from build123d import *

# Parameters (mm, degrees)
SKETCH1_W           = 140
SKETCH1_H           = 140
BOSS_EXTRUDE1_DEPTH = 34
SKETCH3_R           = 8
CUT_EXTRUDE3_DEPTH  = 105.670912865
CHAMFER1_SIZE       = 5
CHAMFER2_SIZE       = 15
CHAMFER3_SIZE       = 40


with BuildPart() as part:
    # Sketch1 → Boss-Extrude1 (new body)
    with BuildSketch(Plane.XY):
        Rectangle(SKETCH1_W, SKETCH1_H)
    extrude(amount=BOSS_EXTRUDE1_DEPTH)

    # Sketch3 → Cut-Extrude3 (cut, through all)
    with BuildSketch(Plane.XY.offset(34)):
        with Locations((0, -50)):
            Circle(SKETCH3_R)
    extrude(amount=-CUT_EXTRUDE3_DEPTH, mode=Mode.SUBTRACT)

    # Chamfer1
    chamfer1_edges = [part.edges().sort_by_distance(p)[0] for p in [
        (-70, 70, 17),
        (70, 70, 17),
    ]]
    chamfer(chamfer1_edges, length=CHAMFER1_SIZE)

    # Chamfer2
    chamfer2_edges = [part.edges().sort_by_distance(p)[0] for p in [
        (0, 70, 34),
    ]]
    chamfer(chamfer2_edges, length=CHAMFER2_SIZE)

    # Chamfer3
    chamfer3_edges = [part.edges().sort_by_distance(p)[0] for p in [
        (70, -70, 17),
        (-70, -70, 17),
    ]]
    chamfer(chamfer3_edges, length=CHAMFER3_SIZE)


solid = part.part
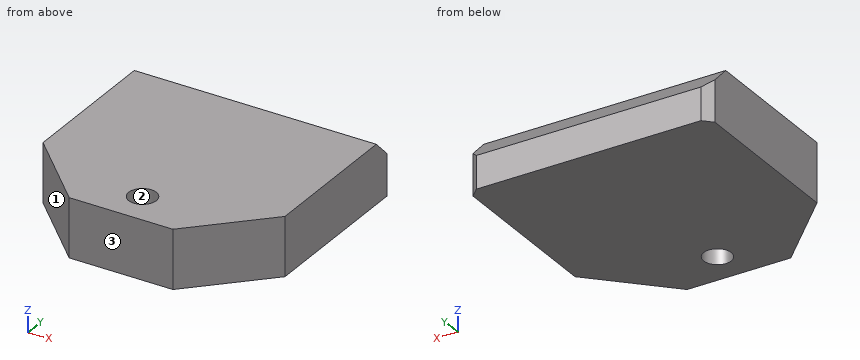
Model file for the job. Use its own axes, mm. Face numbers are marked on the shaded views. Give positions to 0.01 mm unless a question says otherwise; leave off trailing zeros. Order: outer loops, then holes, each group sorted by start corner. A loop starts at its lowest first (then second) coordinate and runs counter-clockwise, first axis right, second up. Notation, with made-up numbers: (86.5, 18.25) - (109.5, 18.25) arc R25 cw to (109.5, 42.25) - close; hole circle Ø6 at (34, 2). An arc over 180 degrees is marked (long way). Return JSON: item names as keys, results as strings.
1) Cut at C-C, the plane y = -50. Give the cut face in (x, z).
Geometry says:
{"outline": "(-50, 0) - (-8, 0) - (-8, 34) - (-50, 34) - close; (8, 0) - (50, 0) - (50, 34) - (8, 34) - close"}
2) Flat gauge pin, fed straight in: P1, Ø18.5, axis at x = 0, y = -50, coming from the -Z side. Where does the tip first touch, or does it go through?
Geometry says:
{"P1": "z = 0"}
3) Cut at A-A, the plane x = 0. Give the cut face in (y, z), plus the area to 3 significant figures.
Geometry says:
{"outline": "(-70, 0) - (-58, 0) - (-58, 34) - (-70, 34) - close; (-42, 0) - (70, 0) - (70, 19) - (55, 34) - (-42, 34) - close", "area": "4,100 mm²"}
4) Cut at B-B, the plane z = 30. Give the cut face in (x, y), plus the area to 3 significant figures.
Geometry says:
{"outline": "(-70, -30) - (-30, -70) - (30, -70) - (70, -30) - (70, 59) - (-70, 59) - close; hole circle Ø16 at (0, -50)", "area": "16,300 mm²"}
5) Probe line 1 (Y direction, x = 0, z = 14); line 2 (Y direction, x = 0, z = 24); line 3 (Y direction, x = 54, z = 12.5). List the from-to ranges inside material, lowest first. Write a range as from..to.
Geometry says:
{"line 1": "-70..-58, -42..70", "line 2": "-70..-58, -42..65", "line 3": "-46..70"}
6) Pull direction X, two halves, no side cores. Call the marked faces 1, 2 and 3: pulls with the +X half, pulls with the -X half, needs draft (parallel to the pull), parting line crosses it, or undercut.
Geometry says:
{"face 1": "pulls with the -X half", "face 2": "undercut", "face 3": "needs draft"}
7) Cut at D-D, the plane z = 16. Give the cut face in (x, y), plus the area to 3 significant figures.
Geometry says:
{"outline": "(-70, -30) - (-30, -70) - (30, -70) - (70, -30) - (70, 65) - (65, 70) - (-65, 70) - (-70, 65) - close; hole circle Ø16 at (0, -50)", "area": "17,800 mm²"}
